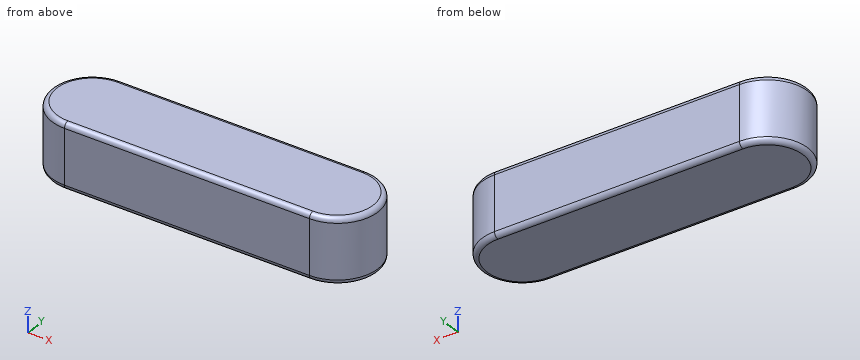
from build123d import *

# Parameters (mm, degrees)
EXTRUDE_523_DEPTH = 8
FILLET_1_R        = 0.6


with BuildPart() as part:
    # 草图1 → Extrude 523 (new body)
    with BuildSketch(Plane.XY):
        with BuildLine():
            Line((-15, 5), (15, 5))
            ThreePointArc((15, 5), (20, 0), (15, -5))
            Line((15, -5), (-15, -5))
            ThreePointArc((-15, -5), (-20, 0), (-15, 5))
        make_face()
    extrude(amount=EXTRUDE_523_DEPTH)

    # 圆角1
    fillet_1_edges = [part.edges().sort_by_distance(p)[0] for p in [
        (20, 0, 8),
        (0, 5, 8),
        (-20, 0, 8),
        (0, 5, 0),
        (20, 0, 0),
        (0, -5, 0),
        (-20, 0, 0),
        (0, -5, 8),
    ]]
    fillet(fillet_1_edges, radius=FILLET_1_R)


solid = part.part
The listing builds one solid part. Answer for the finished solid, in the listing's coordinates (mm). Round coordinates to 2 decimals unless told otherwise and drop trailing zeros. Write each loop counter-clockwise with the first axis right and the second up, starting at its lowest first coordinate (ties: lowest second). Pieces come first, ordered by that corner, then holes. Notation, with made-up numbers: M 13,-21.75 L 68,-21.75 A18 cw 68,6.25 Z; hole C 74,19.5 d5. An arc over 180 degrees is marked long. Write each question's results on one line, items separated by ' | '. Start each with the question number.
Item 1: Find section A-A on z = 3.75. Write down the section's boundary in (x, y), and give its area (3 significant figures).
Item 2: Straight lines are drawn through the part: probe 1 along Y at (x, z) = (-13.5, 7.5); probe 2 along X at (y, z) = (0.25, 6.5); probe 3 along X at (y, z) = (1, 7.5). For each, find the intervals that lie inside material, in ascending order.
Item 3: Given pin 1 Ø1 at (y, z) = (1.5, 6.5) entering from -X; pin 2 Ø1.5 at (y, z) = (-3.5, 2.5) entering from +X, each flat-ended and moving along its own axis, determine where each tip first touches the part or whether it passes through.
Answer block:
1) outline: M -15,-5 L 15,-5 A5 ccw 15,5 L -15,5 A5 ccw Z | area: 379 mm²
2) probe 1: y = -4.99 to 4.99 | probe 2: x = -19.99 to 19.99 | probe 3: x = -19.89 to 19.89
3) pin 1: stops at x = -19.9 | pin 2: stops at x = 19.18
